Read the model definition and answer for the solid it produces. Units are mm, in the model's axes. A direction names the side the tool comes from. Coordinates: 2 decimals unless noted, no trailing zeros. Write each loop counter-clockwise with the first axis right and the second up, starting at its lowest first coordinate (ties: lowest second). Pieces come first, ordered by that corner, then holes.
Item 1: Determine the mould class of faces 5 (the face through (35, 15, 53)), 6 (the face through (35, 50, 10)), 7 (the face through (70, 19, 27)) for opening direction X: released by +X, released by -X, zero draft, split by the parting line, or undercut.
Item 2: Each of these flat-tipped pins is pushed along its axis until it touches: P1, Ø4, axis at y = 6.5, z = 58, coming from the -X side; P2, Ø7.5, axis at x = 50, z = 30, coming from the +Y side; P3, Ø9, axis at x = 35, z = 42.5, coming from the -Y side; P4, Ø3, axis at x = 41.5, y = 3.5, coming from the +Z side. Where does it stop, or does it pass through?
Item 3: Section C-C (z = 56) is taken. Give the vertices of the cut face in (x, y).
Item 4: Straight lines are drawn through the part: probe 1 along Z at (x, y) = (44, 7); probe 2 along Y at (x, z) = (43, 27.5); probe 3 along Z at (x, y) = (31.5, 12). For each, find the intervals that lie inside material, in ascending order.
Item 5: Section B-B (y = 12) is taken. Give the vertices of the cut face in (x, z).
Item 6: Section D-D (x = 38.5) is taken. Give the vertices of the cut face in (y, z).
Item 7: Section A-A (x = 52.5) is taken. Give the vertices of the cut face in (y, z), then the cut area to 3 significant figures.
Item 8: A tool of negligible diameter and unlimited length cuts with its end or side. For faces 1 (the face through (20, 9, 57)), 2 (the face through (35, 10, 32)), 3 (the face through (35, 37, 35)), 4 (the face through (17.745, 27.605, 52.745)), from which of +Z, -Z, +X, -X, +Y, -Y can it reach the whole face along a straight path? Write none if from no direction.
from build123d import *

# Parameters (mm, degrees)
BASE_BLOCK_SKETCH_W  = 70
BASE_BLOCK_SKETCH_H  = 50
BASE_BLOCK_DEPTH     = 15
PAD_SKETCH_W         = 70
PAD_SKETCH_H         = 50
PAD_5MM_DEPTH        = 5
STEPPED_BODY_DEPTH   = 70
ANGLED_WEDGE_DEPTH   = 35
FRONT_SLOT_CUT_DEPTH = 35


with BuildPart() as part:
    # Base Block Sketch → Base Block (new body)
    with BuildSketch(Plane.XY):
        with Locations((35, 25)):
            Rectangle(BASE_BLOCK_SKETCH_W, BASE_BLOCK_SKETCH_H)
    extrude(amount=BASE_BLOCK_DEPTH)

    # Pad Sketch → Pad 5mm (add)
    with BuildSketch(Plane.XY.offset(15)):
        with Locations((35, 25)):
            Rectangle(PAD_SKETCH_W, PAD_SKETCH_H)
    extrude(amount=PAD_5MM_DEPTH)

    # Stepped Profile Sketch → Stepped Body (add)
    with BuildSketch(Plane.ZY):
        Polygon((20, 40), (35, 40), (35, 20), (70, 20), (70, 0), (50, 0), (50, 10), (20, 10), align=None)
    extrude(amount=-STEPPED_BODY_DEPTH)

    # Wedge Sketch → Angled Wedge (add)
    with BuildSketch(Plane.XY.offset(70)):
        Polygon((35, 35), (0, 20), (70, 20), align=None)
    extrude(amount=-ANGLED_WEDGE_DEPTH)

    # Slot Cut Sketch → Front Slot Cut (cut)
    with BuildSketch(Plane.XY.offset(70)):
        Polygon((35, 0), (20, 0), (20, 15), (50, 15), (50, 0), align=None)
    extrude(amount=-FRONT_SLOT_CUT_DEPTH, mode=Mode.SUBTRACT)


solid = part.part
Established:
1. face 5: undercut
1. face 6: zero draft
1. face 7: released by +X
2. P1: stops at x = 0
2. P2: stops at y = 40
2. P3: stops at y = 15
2. P4: stops at z = 20
3. outline: (0, 0) - (20, 0) - (20, 15) - (50, 15) - (50, 0) - (70, 0) - (70, 20) - (35, 35) - (0, 20) - close
4. probe 1: z = 0 to 20
4. probe 2: y = 10 to 40
4. probe 3: z = 0 to 35
5. outline: (0, 0) - (70, 0) - (70, 70) - (50, 70) - (50, 35) - (20, 35) - (20, 70) - (0, 70) - close
6. outline: (0, 0) - (50, 0) - (50, 20) - (40, 20) - (40, 35) - (33.5, 35) - (33.5, 70) - (15, 70) - (15, 35) - (10, 35) - (10, 20) - (0, 20) - close
7. outline: (0, 0) - (50, 0) - (50, 20) - (40, 20) - (40, 35) - (27.5, 35) - (27.5, 70) - (0, 70) - (0, 50) - (10, 50) - (10, 20) - (0, 20) - close
7. area: 2,260 mm2
8. face 1: +Z, -Y
8. face 2: +X, -X, -Y
8. face 3: +Z, +Y
8. face 4: +Z, -X, +Y
